```python
from build123d import *

# Parameters (mm, degrees)
SKETCH_1_W      = 370
SKETCH_1_H      = 34
SKETCH_1_R      = 5.5
EXTRUDE_1_DEPTH = 10


with BuildPart() as part:
    # 草图1 → 凸台-拉伸1 (new body)
    with BuildSketch(Plane.XY):
        Rectangle(SKETCH_1_W, SKETCH_1_H)
        with Locations((165, -5)):
            Circle(SKETCH_1_R, mode=Mode.SUBTRACT)
        with Locations((55, -5)):
            Circle(SKETCH_1_R, mode=Mode.SUBTRACT)
        with Locations((-55, -5)):
            Circle(SKETCH_1_R, mode=Mode.SUBTRACT)
        with Locations((-165, -5)):
            Circle(SKETCH_1_R, mode=Mode.SUBTRACT)
    extrude(amount=EXTRUDE_1_DEPTH)


solid = part.part
```
The listing builds one solid part. Answer for the finished solid, in the listing's coordinates (mm). Give positions to 0.01 mm unless a question says otherwise; leave off trailing zeros. Loops run counter-clockwise (first coordinate to the right, second up) from the corner with the lowest first, then second, coordinate; pieces in that order, holes last. Notation, with made-up numbers: (-7.5, 67.25) - (46.5, 67.25) arc R15 cw to (46.5, 73.25) - close; hole circle Ø9 at (-3, 63). An arc over 180 degrees is marked (long way). Return JSON: item names as keys, results as strings. Group by question number.
1. Determine the mould class of faces 1 (the flat face through (-3, 17, 5)), 2 (the flat face through (-185, 0, 5)), 3 (the cylindrical face through (-170.495, -4.758, 4.93)) for opening direction Y: pulls with the +Y half, pulls with the -Y half, needs draft (parallel to the pull), parting line crosses it, or undercut.
2. Find section C-C (x = -55). Write down the section's boundary in (y, z), then the cut area to 3 significant figures.
3. Find section A-A (y = -5). Write down the section's boundary in (x, z), then the cut area to 3 significant figures.
4. Straight lines are drawn through the part: line 1 (X direction, y = -2, z = 4); line 2 (Y direction, x = 165, z = 4.75); line 3 (X direction, y = -1, z = 9.5). For each, find the intervals that lie inside material, in ascending order. Write a range as [from, to].
5. Find section B-B (z = 3). Write down the section's boundary in (x, y), then the cut area to 3 significant figures.
Verdict:
{
 "1": {"face 1": "pulls with the +Y half", "face 2": "needs draft", "face 3": "undercut"},
 "2": {"outline": "(-17, 0) - (-10.5, 0) - (-10.5, 10) - (-17, 10) - close; (0.5, 0) - (17, 0) - (17, 10) - (0.5, 10) - close", "area": "230 mm^2"},
 "3": {"outline": "(-185, 0) - (-170.5, 0) - (-170.5, 10) - (-185, 10) - close; (-159.5, 0) - (-60.5, 0) - (-60.5, 10) - (-159.5, 10) - close; (-49.5, 0) - (49.5, 0) - (49.5, 10) - (-49.5, 10) - close; (60.5, 0) - (159.5, 0) - (159.5, 10) - (60.5, 10) - close; (170.5, 0) - (185, 0) - (185, 10) - (170.5, 10) - close", "area": "3,260 mm^2"},
 "4": {"line 1": "x = [-185, -169.61], [-160.39, -59.61], [-50.39, 50.39], [59.61, 160.39], [169.61, 185]", "line 2": "y = [-17, -10.5], [0.5, 17]", "line 3": "x = [-185, -168.77], [-161.23, -58.77], [-51.23, 51.23], [58.77, 161.23], [168.77, 185]"},
 "5": {"outline": "(-185, -17) - (185, -17) - (185, 17) - (-185, 17) - close; hole circle Ø11 at (-165, -5); hole circle Ø11 at (-55, -5); hole circle Ø11 at (55, -5); hole circle Ø11 at (165, -5)", "area": "12,200 mm^2"}
}
